Source: CAD feature listing. Evaluate the final solid. Frame: model axes, mm. A direction names the side the tool comes from. Round coordinates to 2 decimals unless told otherwise and drop trailing zeros. Write each loop counter-clockwise with the first axis right and the second up, starting at its lowest first coordinate (ties: lowest second). Pieces come first, ordered by that corner, then holes.
from build123d import *

# Parameters (mm, degrees)
BOSS_EXTRUDE2_DEPTH                                  = 110
CBORE_FOR_M3_SLOTTED_CHEESE_HEAD_SCREWS2_D           = 3.4
CBORE_FOR_M3_SLOTTED_CHEESE_HEAD_SCREWS2_CBORE_D     = 6
CBORE_FOR_M3_SLOTTED_CHEESE_HEAD_SCREWS2_CBORE_DEPTH = 3.4
CBORE_FOR_M3_SLOTTED_CHEESE_HEAD_SCREWS3_D           = 3.4
CBORE_FOR_M3_SLOTTED_CHEESE_HEAD_SCREWS3_CBORE_D     = 6
CBORE_FOR_M3_SLOTTED_CHEESE_HEAD_SCREWS3_CBORE_DEPTH = 3.4
F_3_0MM_DOWEL_HOLE1_D                                = 3
CUT_EXTRUDE1_DEPTH                                   = 111.480767557
CHAMFER1_SIZE                                        = 0.5


with BuildPart() as part:
    # Sketch4 → Boss-Extrude2 (new body)
    with BuildSketch(Plane.XY):
        Polygon((0, 0), (9, 0), (9, 3.5), (8, 3.5), (8, 5), (0, 5), (0, 3.5), align=None)
    extrude(amount=BOSS_EXTRUDE2_DEPTH)

    # CBORE for M3 Slotted cheese head screws2 (through all)
    with Locations(Plane(origin=(0, 5, 0), x_dir=(1, 0, 0), z_dir=(0, 1, 0))):
        with Locations((4, -10), (4, -100)):
            CounterBoreHole(CBORE_FOR_M3_SLOTTED_CHEESE_HEAD_SCREWS2_D / 2, CBORE_FOR_M3_SLOTTED_CHEESE_HEAD_SCREWS2_CBORE_D / 2, CBORE_FOR_M3_SLOTTED_CHEESE_HEAD_SCREWS2_CBORE_DEPTH)

    # CBORE for M3 Slotted cheese head screws3 (through all)
    with Locations(Plane.XZ):
        with Locations((4, 90), (4, 20)):
            CounterBoreHole(CBORE_FOR_M3_SLOTTED_CHEESE_HEAD_SCREWS3_D / 2, CBORE_FOR_M3_SLOTTED_CHEESE_HEAD_SCREWS3_CBORE_D / 2, CBORE_FOR_M3_SLOTTED_CHEESE_HEAD_SCREWS3_CBORE_DEPTH)

    # Ø3.0mm dowel hole1 (through all)
    with Locations(Plane.XZ):
        with Locations((4, 80), (4, 30)):
            Hole(F_3_0MM_DOWEL_HOLE1_D / 2)

    # Sketch11 → Cut-Extrude1 (cut, through all)
    with BuildSketch(Plane.XZ):
        with BuildLine():
            Line((2.5, 78.5), (2.5, 81.5))
            ThreePointArc((2.5, 81.5), (4, 83), (5.5, 81.5))
            Line((5.5, 81.5), (5.5, 78.5))
            ThreePointArc((5.5, 78.5), (4, 77), (2.5, 78.5))
        make_face()
    extrude(amount=-CUT_EXTRUDE1_DEPTH, mode=Mode.SUBTRACT)

    # Chamfer1
    chamfer1_edges = [part.edges().sort_by_distance(p)[0] for p in [
        (0, 5, 55),
        (8, 5, 55),
        (9, 1.75, 110),
        (9, 3.5, 55),
        (9, 0, 55),
        (0, 0, 55),
        (8.5, 3.5, 110),
        (8, 4.25, 110),
        (4, 5, 110),
        (0, 2.5, 110),
        (0, 2.5, 0),
        (4, 5, 0),
        (8, 4.25, 0),
        (8.5, 3.5, 0),
        (4.5, 0, 110),
        (9, 1.75, 0),
        (4.5, 0, 0),
    ]]
    chamfer(chamfer1_edges, length=CHAMFER1_SIZE)


solid = part.part
1) Section query C-C on z = 42. Return the cut outline in (x, y).
Taken from the geometry:
outline: (0, 0.5) - (0.5, 0) - (8.5, 0) - (9, 0.5) - (9, 3) - (8.5, 3.5) - (8, 3.5) - (8, 4.5) - (7.5, 5) - (0.5, 5) - (0, 4.5) - close
2) Section query B-B on z = 30. Return the cut outline in (x, y), then the cut area to 3 significant figures.
Taken from the geometry:
outline: (0, 0.5) - (0.5, 0) - (2.5, 0) - (2.5, 5) - (0.5, 5) - (0, 4.5) - close; (5.5, 0) - (8.5, 0) - (9, 0.5) - (9, 3) - (8.5, 3.5) - (8, 3.5) - (8, 4.5) - (7.5, 5) - (5.5, 5) - close
area: 27.9 mm2
3) Pull-direction query (X, two-part tool) for faces 1 (the face through (4.37, 4.21, 88.34)), 2 (the face through (4, 3, 0)), 3 (the face through (9, 2, 54)); classes: released by +X, released by -X, zero draft, split by the parting line, or undercut.
Taken from the geometry:
face 1: undercut
face 2: zero draft
face 3: released by +X
4) Contact query for flat-ended pins moving along their axis: P1, Ø5, axis at x = 4, z = 10, coming from the +Y side; P2, Ø3, axis at x = 4, z = 89.5, coming from the -Y side. Output: stop coordinate, or through.
Taken from the geometry:
P1: stops at y = 1.6
P2: stops at y = 3.4
5) Section query A-A on z = 10. Return the cut outline in (x, y).
Taken from the geometry:
outline: (0, 0.5) - (0.5, 0) - (2.3, 0) - (2.3, 1.6) - (1, 1.6) - (1, 5) - (0.5, 5) - (0, 4.5) - close; (5.7, 0) - (8.5, 0) - (9, 0.5) - (9, 3) - (8.5, 3.5) - (8, 3.5) - (8, 4.5) - (7.5, 5) - (7, 5) - (7, 1.6) - (5.7, 1.6) - close
6) Material intervals for line 1 (Z direction, x = 2.25, y = 3); line 2 (X direction, y = 4.25, z = 62.5); line 3 (Y direction, x = 8.5, z = 105), sorted ascending.
Taken from the geometry:
line 1: z = 0 to 7.56, 12.44 to 17.56, 22.44 to 87.56, 92.44 to 97.56, 102.44 to 110
line 2: x = 0 to 8
line 3: y = 0 to 3.5
7) Reachability of faces 4 (the face through (4, 3, 110)), 5 (the face through (4, 2, 77)), 6 (the face through (6, 3.4, 90)), 7 (the face through (6, 1.6, 100)), 8 (the face through (4, 5, 54)) from +Z, -Z, +X, -X, +Y, -Y: full face, straight path, thin tool, end or side. Return the list, or none.
Taken from the geometry:
face 4: +Z, +X, -X, +Y, -Y
face 5: +Y, -Y
face 6: -Y
face 7: +Y
face 8: +Z, -Z, +X, -X, +Y
8) Section query D-D on x = 4.25. State how many separate pieces and enclosed holes the cut face has, then the cut area to 3 significant figures.
Taken from the geometry:
separate pieces: 7
enclosed holes: 0
area: 402 mm2
